The listing builds one solid part. Answer for the finished solid, in the listing's coordinates (mm). A direction names the side the tool comes from. Coordinates: 2 decimals unless noted, no trailing zeros. Order: outer loops, then holes, each group sorted by start corner. A loop starts at its lowest first (then second) coordinate and runs counter-clockwise, first axis right, second up. Notation, with made-up numbers: M 56,-39.5 L 104,-39.5 A7 ccw 104,-34.5 Z; hole C 1.25,47 d7. An arc over 180 degrees is marked long. One line per item, written item: value. Start each with the question number.
Q1. The part is cut by section B-B on z = 45. Give the vertices of the cut face in (x, y).
Q2. For faces 1 (the flat face through (-5, 6, 67)), 2 (the flat face through (-3, -5, 90)), 3 (the cylindrical face through (-10.017, 0.13, 97.535)), determine the directions among +Z, -Z, +X, -X, +Y, -Y from which every point of the face is accessible in a straight line to the end or side of a thin tool.
Q3. Straight lines are drawn through the part: line 1 along Y through (x, z) = (-3, 87.55); line 2 along Y through (x, z) = (-3, 94.25); line 3 along Z through (x, y) = (-7, -3.75). For each, find the intervals that lie inside material, in ascending order. Write a range as [from, to].
Q4. Determine the mould class of faces 4 (the flat face through (-8, 0, 20)), 5 (the cylindrical face through (5, 1.6, 9.9)), 6 (the flat face through (1, 0, 100)), 7 (the cylindrical face through (-3.45, 6.48, 91.43)) for opening direction Z: pulls with the +Z half, pulls with the -Z half, needs draft (parallel to the pull), parting line crosses it, or undercut.
Q5. The part is cut by section C-C on z = 35. Give the vertices of the cut face in (x, y), then the cut area to 3 significant figures.
Q6. The part is cut by section A-A on z = 11. Give the vertices of the cut face in (x, y).
Q7. Each of these flat-tipped pins is pushed along its axis until it touches: pin 1 Ø2 at (x, z) = (1.5, 32) entering from +Y; pin 2 Ø6.5 at (x, y) = (-5, 0.5) entering from +Z; pin 3 Ø12 at (y, z) = (-4.5, 28.5) entering from -X; pin 4 Ø5.5 at (x, z) = (-5.5, 57) entering from -Y. Where does it stop, or does it pass through?
```python
from build123d import *

# Parameters (mm, degrees)
SKETCH1_R                  = 11
BOSS_EXTRUDE1_DEPTH        = 100
CUT_EXTRUDE1_DEPTH         = 102.202766761
SKETCH3_R                  = 2
CUT_EXTRUDE2_DEPTH         = 60
CUT_EXTRUDE3_START         = -15
SKETCH4_W                  = 13.898015679
SKETCH4_H                  = 8
CUT_EXTRUDE3_DEPTH         = 65
CUT_EXTRUDE4_DEPTH         = 102.867561078
CUT_EXTRUDE4_DEPTH_BACK    = 102.867561078
SKETCH5_W                  = 12
SKETCH5_H                  = 10
M8_TAPPED_HOLE1_D          = 6.8
M8_TAPPED_HOLE1_DEPTH      = 10
M8_TAPPED_HOLE1_TIP        = 2.042926105
CUT_EXTRUDE5_START         = -3
SKETCH8_R                  = 1.5
CUT_EXTRUDE5_DEPTH         = 105.867561078
CUT_EXTRUDE6_DEPTH         = 102.867561078
CUT_EXTRUDE7_DEPTH         = 102.316336294
CUT_EXTRUDE7_DEPTH_BACK    = 102.316336294
M12X1_5_TAPPED_HOLE1_D     = 10.5
M12X1_5_TAPPED_HOLE1_DEPTH = 19.5
M12X1_5_TAPPED_HOLE1_TIP   = 3.15451825
SKETCH12_R                 = 2.5
BOSS_EXTRUDE2_DEPTH        = 2.2
BOSS_EXTRUDE3_START        = 2.2
SKETCH13_R                 = 2.5
BOSS_EXTRUDE3_DEPTH        = 2.2
SKETCH14_R                 = 3.5
CUT_EXTRUDE8_DEPTH         = 40
SKETCH15_R                 = 14.729549922
SKETCH15_R_2               = 10.018203868
CUT_EXTRUDE9_DEPTH         = 5


with BuildPart() as part:
    # Sketch1 → Boss-Extrude1 (new body)
    with BuildSketch(Plane.XY):
        Circle(SKETCH1_R)
    extrude(amount=BOSS_EXTRUDE1_DEPTH)

    # Sketch2 → Cut-Extrude1 (cut, through all)
    with BuildSketch(Plane.XY.offset(100)):
        with BuildLine():
            Line((-7.549834435, 8), (7.549834435, 8))
            ThreePointArc((7.549834435, 8), (0, 11), (-7.549834435, 8))
        make_face()
        with BuildLine():
            Line((-7.549834435, -8), (7.549834435, -8))
            ThreePointArc((7.549834435, -8), (0, -11), (-7.549834435, -8))
        make_face()
    extrude(amount=-CUT_EXTRUDE1_DEPTH, mode=Mode.SUBTRACT)

    # Sketch3 → Cut-Extrude2 (cut)
    with BuildSketch(Plane.XY.offset(100)):
        with Locations((-3, 0)):
            Circle(SKETCH3_R)
    extrude(amount=-CUT_EXTRUDE2_DEPTH, mode=Mode.SUBTRACT)

    # Sketch4 → Cut-Extrude3 (cut)
    with BuildSketch(Plane.XY.offset(100).offset(CUT_EXTRUDE3_START)):
        with Locations((-5.94900784, 0)):
            Rectangle(SKETCH4_W, SKETCH4_H)
    extrude(amount=-CUT_EXTRUDE3_DEPTH, mode=Mode.SUBTRACT)

    # Sketch5 → Cut-Extrude4 (cut, two sides: drawn at the far end of the back side and taken through both)
    with BuildSketch(Plane(origin=(0, -8, 0), x_dir=(-1, 0, 0), z_dir=(0, -1, 0)).offset(-CUT_EXTRUDE4_DEPTH_BACK)):
        with Locations((-11, -100)):
            Rectangle(SKETCH5_W, SKETCH5_H)
    extrude(amount=CUT_EXTRUDE4_DEPTH + CUT_EXTRUDE4_DEPTH_BACK, mode=Mode.SUBTRACT)

    # M8 Tapped Hole1
    with Locations(Plane(origin=(-3, -0.07100101, 100), x_dir=(1, 0, 0), z_dir=(0, 0, 1))):
        with Locations((0, 0)):
            Hole(M8_TAPPED_HOLE1_D / 2, depth=M8_TAPPED_HOLE1_DEPTH)
            with Locations((0, 0, -(M8_TAPPED_HOLE1_DEPTH + M8_TAPPED_HOLE1_TIP / 2))):  # 118° drill point
                Cone(0, M8_TAPPED_HOLE1_D / 2, M8_TAPPED_HOLE1_TIP, mode=Mode.SUBTRACT)

    # Sketch8 → Cut-Extrude5 (cut)
    with BuildSketch(Plane(origin=(0, -8, 0), x_dir=(-1, 0, 0), z_dir=(0, -1, 0)).offset(CUT_EXTRUDE5_START)):
        with Locations(Location((3, -90, 0), (0, 0, 270))):
            Circle(SKETCH8_R)
    cut_extrude5 = extrude(amount=CUT_EXTRUDE5_DEPTH, mode=Mode.SUBTRACT)

    # Mirror3: Cut-Extrude5 across plane
    add(cut_extrude5.mirror(Plane.ZX), mode=Mode.SUBTRACT)

    # Sketch9 → Cut-Extrude6 (cut, through all)
    with BuildSketch(Plane(origin=(0, -8, 0), x_dir=(-1, 0, 0), z_dir=(0, -1, 0))):
        with BuildLine():
            Line((2.5, -30), (2.5, -25))
            ThreePointArc((2.5, -25), (4, -23.5), (5.5, -25))
            Line((5.5, -25), (5.5, -30))
            ThreePointArc((5.5, -30), (4, -31.5), (2.5, -30))
        make_face()
    extrude(amount=-CUT_EXTRUDE6_DEPTH, mode=Mode.SUBTRACT)

    # Sketch10 → Cut-Extrude7 (cut, two sides: drawn at the far end of the back side and taken through both)
    with BuildSketch(Plane(origin=(0, 4, 0), x_dir=(-1, 0, 0), z_dir=(0, -1, 0)).offset(-CUT_EXTRUDE7_DEPTH_BACK)):
        with BuildLine():
            Line((2, -67), (19.82874578, -67))
            Line((19.82874578, -67), (19.82874578, -61))
            Line((19.82874578, -61), (2, -61))
            ThreePointArc((2, -61), (0.585786438, -61.585786438), (0, -63))
            Line((0, -63), (0, -65))
            ThreePointArc((0, -65), (0.585786438, -66.414213562), (2, -67))
        make_face()
    extrude(amount=CUT_EXTRUDE7_DEPTH + CUT_EXTRUDE7_DEPTH_BACK, mode=Mode.SUBTRACT)

    # M12x1.5 Tapped Hole1
    with Locations(Plane(origin=(0, 0, 0), x_dir=(-1, 0, 0), z_dir=(0, 0, -1))):
        with Locations((0, 0)):
            Hole(M12X1_5_TAPPED_HOLE1_D / 2, depth=M12X1_5_TAPPED_HOLE1_DEPTH)
            with Locations((0, 0, -(M12X1_5_TAPPED_HOLE1_DEPTH + M12X1_5_TAPPED_HOLE1_TIP / 2))):  # 118° drill point
                Cone(0, M12X1_5_TAPPED_HOLE1_D / 2, M12X1_5_TAPPED_HOLE1_TIP, mode=Mode.SUBTRACT)

    # Sketch12 → Boss-Extrude2 (add)
    with BuildSketch(Plane.XZ.offset(8)):
        with Locations(Location((-3, 40, 0), (0, 0, 90))):
            Circle(SKETCH12_R)
    extrude(amount=BOSS_EXTRUDE2_DEPTH)

    # Sketch13 → Boss-Extrude3 (add)
    with BuildSketch(Plane(origin=(0, 8, 0), x_dir=(1, 0, 0), z_dir=(0, 1, 0)).offset(BOSS_EXTRUDE3_START)):
        with Locations(Location((-3, -40, 0), (0, 0, 270))):
            Circle(SKETCH13_R)
    extrude(amount=-BOSS_EXTRUDE3_DEPTH)

    # Sketch14 → Cut-Extrude8 (cut)
    with BuildSketch(Plane(origin=(0, 0, 0), x_dir=(-1, 0, 0), z_dir=(0, 0, -1))):
        Circle(SKETCH14_R)
    extrude(amount=-CUT_EXTRUDE8_DEPTH, mode=Mode.SUBTRACT)

    # Sketch15 → Cut-Extrude9 (cut)
    with BuildSketch(Plane.XY.offset(100)):
        Circle(SKETCH15_R)
        Circle(SKETCH15_R_2, mode=Mode.SUBTRACT)
    extrude(amount=-CUT_EXTRUDE9_DEPTH, mode=Mode.SUBTRACT)


solid = part.part
```
Output:
1. outline: M -10.25,-4 A11 ccw -7.55,-8 L 7.55,-8 A11 ccw 7.55,8 L -7.55,8 A11 ccw -10.25,4 L 1,4 L 1,-4 Z
2. face 1: -X, +Y, -Y
2. face 2: -Y
2. face 3: +Z, -X
3. line 1: y = [-8, -2], [2, 8]
3. line 2: y = [-8, -3.47], [3.33, 8]
3. line 3: z = [0, 20], [85, 100]
4. face 4: undercut
4. face 5: needs draft
4. face 6: pulls with the +Z half
4. face 7: undercut
5. outline: M -10.25,-4 A11 ccw -7.55,-8 L 7.55,-8 A11 ccw 7.55,8 L -7.55,8 A11 ccw -10.25,4 L 1,4 L 1,3.35 A3.5 cw 1,-3.35 L 1,-4 Z
5. area: 212 mm^2
6. outline: M -7.55,-8 L 7.55,-8 A11 ccw 7.55,8 L -7.55,8 A11 ccw Z; hole C 0,0 d10.5
7. pin 1: stops at y = 8
7. pin 2: stops at z = 100
7. pin 3: stops at x = -10.25
7. pin 4: stops at y = -8
